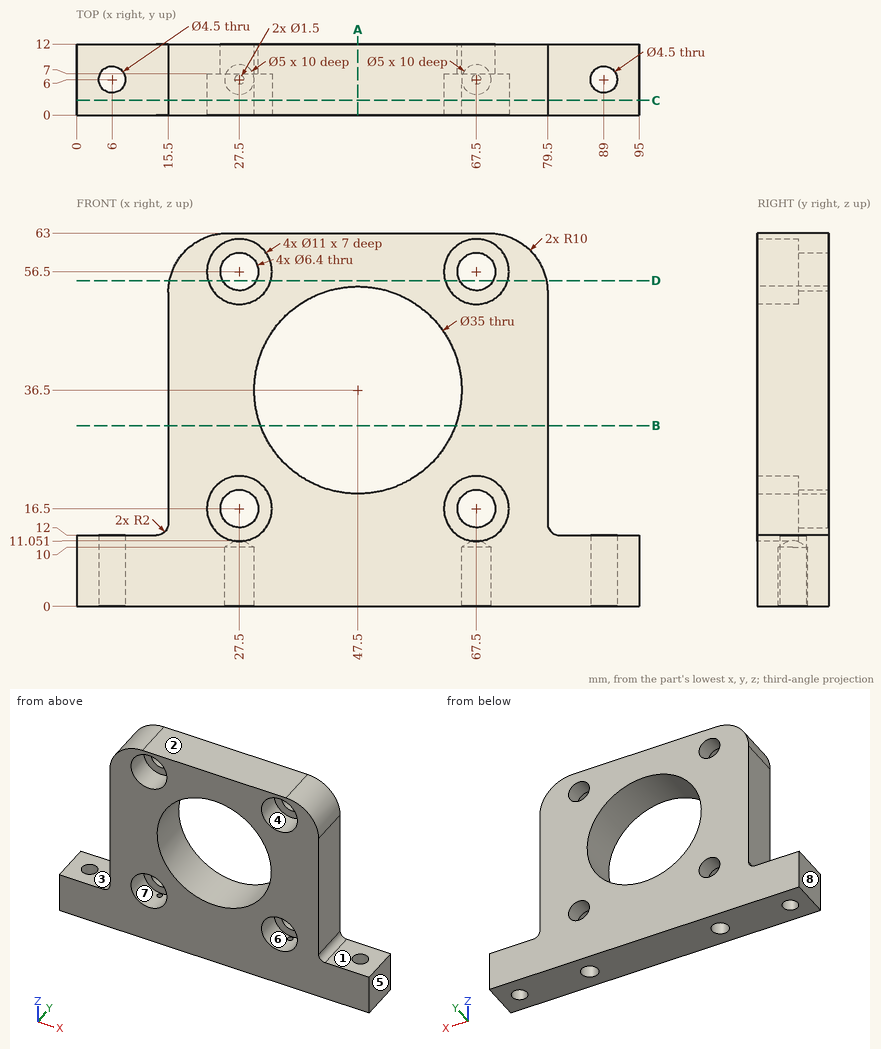
Could you check a few things on this drawing? It's one solid part, dimensions in mm from its lowest x, y, z. A direction names the side the tool comes from. Coordinates: 2 decimals unless noted, no trailing zeros. Order: outer loops, then holes, each group sorted by start corner. A loop starts at its lowest first (then second) coordinate and runs counter-clockwise, first axis right, second up.
1) We'd pull the mould along X, two halves only. Please class the marked faces 5, 6, 7 and 8: +X half, -X half, draft (parallel to the pull), parting line (faces both ways), or undercut.
2) Will these pins go through, and if not, where does the flat tip stop? pin 1 (3 mm diameter, centred on y = 9.5, z = 39, fed in from -X); pin 2 (2.5 mm diameter, centred on x = 89, y = 6, fed in from +Z); pin 3 (6 mm diameter, centred on x = 88, y = 7.5, fed in from +Z); pin 4 (3 mm diameter, centred on x = 27.5, y = 6, fed in from -Z).
3) I need wall thicknesses on line 1 (Z direction, x = 27.5, y = 10.5); line 2 (X direction, y = 4.25, z = 16.5); line 3 (X direction, y = 3.25, z = 56.5). Which ranges of each line are inside material? Lowest first, please.
4) Which directions (+Z, -Z, +X, -X, +Y, -Y) give clear straight access to the entire face, cutting with the end or side of a thin tool? Please do the marked faces 1, 2, 3 and 4.
5) Imagine slicing it at B-B on z = 30.5. List the corners of the cut face in (x, y) for me.
6) Imagine slicing it at C-C on y = 2.5. List the corners of the cut face in (x, z) for me, and give its area (3 significant figures).
7) Imagine slicing it at D-D on z = 55. List the corners of the cut face in (x, y) for me.
8) Imagine slicing it at A-A on x = 47.5. List the corners of the cut face in (y, z) for me, and give its area (3 significant figures).
Response values:
1. face 5: +X half
1. face 6: undercut
1. face 7: undercut
1. face 8: -X half
2. pin 1: stops at x = 15.5
2. pin 2: passes through
2. pin 3: stops at z = 12
2. pin 4: stops at z = 10.6
3. line 1: z = 0 to 13.3, 19.7 to 53.3, 59.7 to 63
3. line 2: x = 15.5 to 22, 33 to 62, 73 to 79.5
3. line 3: x = 16.13 to 22, 33 to 62, 73 to 78.87
4. face 1: +Z, +X, +Y, -Y
4. face 2: +Z, +X, -X, +Y, -Y
4. face 3: +Z, -X, +Y, -Y
4. face 4: -Y
5. outline: (15.5, 0) - (31.06, 0) - (31.06, 12) - (15.5, 12) - close; (63.94, 0) - (79.5, 0) - (79.5, 12) - (63.94, 12) - close
6. outline: (0, 0) - (95, 0) - (95, 12) - (81.5, 12) arc R2 cw to (79.5, 14) - (79.5, 53) arc R10 ccw to (69.5, 63) - (25.5, 63) arc R10 ccw to (15.5, 53) - (15.5, 14) arc R2 cw to (13.5, 12) - (0, 12) - close; hole circle Ø11 at (27.5, 16.5); hole circle Ø11 at (27.5, 56.5); hole circle Ø35 at (47.5, 36.5); hole circle Ø11 at (67.5, 16.5); hole circle Ø11 at (67.5, 56.5)
6. area: 3,020 mm2
7. outline: (15.7, 0) - (22.21, 0) - (22.21, 7) - (24.67, 7) - (24.67, 12) - (15.7, 12) - close; (30.33, 7) - (32.79, 7) - (32.79, 0) - (62.21, 0) - (62.21, 7) - (64.67, 7) - (64.67, 12) - (30.33, 12) - close; (70.33, 7) - (72.79, 7) - (72.79, 0) - (79.3, 0) - (79.3, 12) - (70.33, 12) - close
8. outline: (0, 0) - (12, 0) - (12, 19) - (0, 19) - close; (0, 54) - (12, 54) - (12, 63) - (0, 63) - close
8. area: 336 mm2
